```python
from build123d import *

# Parameters (mm, degrees)
SKETCH1_R           = 27.5
SKETCH1_R_2         = 17.5
BOSS_EXTRUDE1_DEPTH = 5
HOLE1_D             = 5
HOLE1_CSINK_D       = 9
HOLE1_CSINK_ANGLE   = 90


with BuildPart() as part:
    # Sketch1 → Boss-Extrude1 (new body)
    with BuildSketch(Plane(origin=(0, 0, 0), x_dir=(1, 0, 0), z_dir=(0, 1, 0))):
        with Locations(Location((0, 0, 0), (0, 0, 270))):
            Circle(SKETCH1_R)
        with Locations(Location((0, 0, 0), (0, 0, 270))):
            Circle(SKETCH1_R_2, mode=Mode.SUBTRACT)
    extrude(amount=BOSS_EXTRUDE1_DEPTH)

    # Hole1 (through all)
    with Locations(Plane(origin=(0, 5, 0), x_dir=(1, 0, 0), z_dir=(0, 1, 0))):
        with Locations((-19.485571585, -11.25), (0, 22.5), (19.485571585, -11.25)):
            CounterSinkHole(HOLE1_D / 2, HOLE1_CSINK_D / 2, counter_sink_angle=HOLE1_CSINK_ANGLE)


solid = part.part
```
Model file for the job. Use its own axes, mm. Give positions to 0.01 mm unless a question says otherwise; leave off trailing zeros. Write each loop counter-clockwise with the first axis right and the second up, starting at its lowest first coordinate (ties: lowest second). Pieces come first, ordered by that corner, then holes. Notation, with made-up numbers: M -36,66.25 L 6,66.25 A23 ccw 6,102.25 Z; hole C 64.25,14 d1. An arc over 180 degrees is marked long. Use a Markdown table: item, result.
1) Cut at D-D (x = -13). List the corners of the cut face in (y, z).
Responses:
| item | result |
|---|---|
| outline | M 0,-24.23 L 5,-24.23 L 5,-11.72 L 0,-11.72 Z; M 0,11.72 L 5,11.72 L 5,24.23 L 0,24.23 Z |
2) Pin check, flat tips, straight feed: pin 1 (8 mm diameter, centred on x = -19.49, z = 11.25, fed in from +Y); pin 2 (3 mm diameter, centred on x = -15.5, y = 2.5, fed in from -Z); pin 3 (1 mm diameter, centred on y = 2.5, z = -17, fed in from +X). Stop position of each tip, or through.
Responses:
| item | result |
|---|---|
| pin 1 | stops at y = 4.5 |
| pin 2 | stops at z = -23.67 |
| pin 3 | stops at x = 22 |
3) Drill centre lines: line 1 (X direction, y = 0.7, z = 11.25); line 2 (Z direction, x = -2.5, y = 4.6); line 3 (X direction, y = 4.4, z = 12.5). Where is each one in solid material? Low to high. Write a range as from..to.
Responses:
| item | result |
|---|---|
| line 1 | x = -25.09..-21.99, -16.99..-13.4, 13.4..16.99, 21.99..25.09 |
| line 2 | z = -27.39..-25.75, -19.25..-17.32, 17.32..27.39 |
| line 3 | x = -24.49..-23.18, -15.79..-12.25, 12.25..15.79, 23.18..24.49 |
4) Cut at C-C (y = 1.8). List the corners of the cut face in (x, z).
Responses:
| item | result |
|---|---|
| outline | C 0,0 d55; hole C -19.49,11.25 d5; hole C 0,0 d35; hole C 0,-22.5 d5; hole C 19.49,11.25 d5 |
5) Pull direction Z, two halves, no side cores. Call faces 1 (the cylindrical face through (-24.397, 2.465, 12.69)), 2 (the flat face through (-18, 0, 0)), 3 (the cylindrical face through (0, 1, -25)), 4 (the cylindrical face through (18.332, 1.479, 13.468)): +Z half, -Z half, draft (parallel to the pull), parting line (faces both ways), or undercut.
Responses:
| item | result |
|---|---|
| face 1 | parting line |
| face 2 | draft |
| face 3 | undercut |
| face 4 | undercut |
6) Cut at B-B (x = 0). List the corners of the cut face in (y, z).
Responses:
| item | result |
|---|---|
| outline | M 0,-27.5 L 5,-27.5 L 5,-27 L 3,-25 L 0,-25 Z; M 0,-20 L 3,-20 L 5,-18 L 5,-17.5 L 0,-17.5 Z; M 0,17.5 L 5,17.5 L 5,27.5 L 0,27.5 Z |
7) Cut at A-A (z = 0). List the corners of the cut face in (x, y).
Responses:
| item | result |
|---|---|
| outline | M -27.5,0 L -17.5,0 L -17.5,5 L -27.5,5 Z; M 17.5,0 L 27.5,0 L 27.5,5 L 17.5,5 Z |
